from build123d import *

# Parameters (mm, degrees)
SKETCH1_W           = 250
SKETCH1_H           = 100
SKETCH2_R           = 225
BOSS_EXTRUDE1_DEPTH = 30
SKETCH3_R           = 125
BOSS_EXTRUDE2_DEPTH = 80
BOSS_EXTRUDE3_DEPTH = 10
CIRPATTERN1_COUNT   = 4


with BuildPart() as part:
    # Sketch1 → Revolve1 (revolve)
    with BuildSketch(Plane.XY, mode=Mode.PRIVATE) as revolve1_sk:
        with Locations((125, 50)):
            Rectangle(SKETCH1_W, SKETCH1_H)
    revolve(revolve1_sk.sketch.rotate(Axis((0, 0, 0), (0, 1, 0)), 90), axis=Axis((0, 0, 0), (0, 1, 0)))

    # Sketch2 → Boss-Extrude1 (add)
    with BuildSketch(Plane(origin=(0, 100, 0), x_dir=(1, 0, 0), z_dir=(0, 1, 0))):
        with Locations(Location((0, 0, 0), (0, 0, 270))):
            Circle(SKETCH2_R)
    extrude(amount=BOSS_EXTRUDE1_DEPTH)

    # Sketch3 → Boss-Extrude2 (add)
    with BuildSketch(Plane(origin=(0, 130, 0), x_dir=(1, 0, 0), z_dir=(0, 1, 0))):
        with Locations(Location((0, 0, 0), (0, 0, 270))):
            Circle(SKETCH3_R)
    extrude(amount=BOSS_EXTRUDE2_DEPTH)

    # Sketch4 → Revolve2 (revolve)
    with BuildSketch(Plane.XY):
        with BuildLine():
            Line((0, 210), (0, 275.518788168))
            ThreePointArc((0, 275.518788168), (70.565061473, 258.146319153), (125, 210))
            Line((125, 210), (0, 210))
        make_face()
    revolve(axis=Axis((0, 210, 0), (0, 1, 0)))

    # Sketch5 → Boss-Extrude3 (add, symmetric)
    with BuildSketch(Plane.XY):
        Polygon((-194.003425054, 130), (-182.358299763, 130), (-182.358299763, 145.262915146), (-182.358299763, 630), (-197.365341888, 630), (-218.16183032, 483.058469024), (-218.16183032, 211.101864805), (-194.003425054, 197.687306821), align=None)
    boss_extrude3 = extrude(amount=BOSS_EXTRUDE3_DEPTH, both=True)

    # CirPattern1: Boss-Extrude3 ×4 about axis
    cirpattern1_axis = Axis((0, 0, 0), (0, 1, 0))
    for i in range(1, CIRPATTERN1_COUNT):
        add(boss_extrude3.rotate(cirpattern1_axis, i * 360 / CIRPATTERN1_COUNT))


solid = part.part
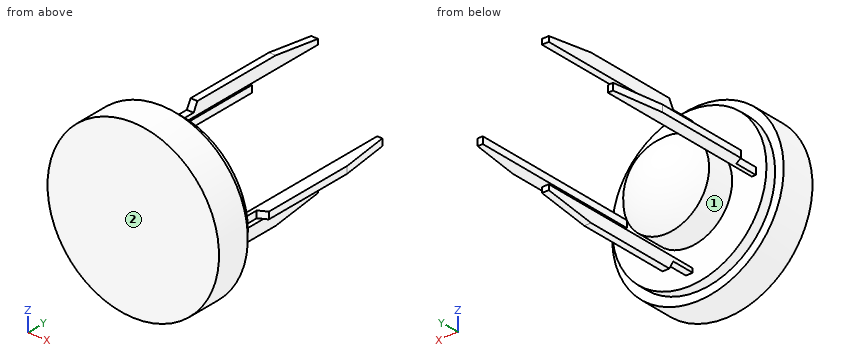
Verification items for the finished model (mm, model axes). Face numbers are marked on the shaded views. A direction names the side the tool comes from. Coordinates: 2 decimals unless noted, no trailing zeros. Write each loop counter-clockwise with the first axis right and the second up, starting at its lowest first coordinate (ties: lowest second). Pieces come first, ordered by that corner, then holes. Notation, with made-up numbers: M -19.75,44.25 L 32.25,44.25 A23 cw 32.25,53.25 Z; hole C 66,-20 d7. An arc over 180 degrees is marked long. Use CSV: the item, a comma, the result in double quotes.
Q1. Section check C-C, the plane z = 0. Enter the section's corners in (x, y).
Computed values:
outline,"M -250,0 L 250,0 L 250,100 L 225,100 L 225,130 L 194,130 L 194,197.69 L 218.16,211.1 L 218.16,483.06 L 197.37,630 L 182.36,630 L 182.36,130 L 125,130 L 125,210 A152 ccw -125,210 L -125,130 L -182.36,130 L -182.36,630 L -197.37,630 L -218.16,483.06 L -218.16,211.1 L -194,197.69 L -194,130 L -225,130 L -225,100 L -250,100 Z"
Q2. Thickness scan on line 1 along Z through (x, y) = (-5.5, 144.5); line 2 along Y through (x, z) = (220, -118); line 3 along Y through (x, z) = (28, 197.5). Record the ranges inside material, lowest first. Write a range as [from, to].
Computed values:
line 1,"[-194, -182.36], [-124.88, 124.88], [182.36, 194]"
line 2,"[0, 100]"
line 3,"[0, 130]"
Q3. Go/stop test with flat-tipped pins: P1, Ø22, axis at x = 0.5, y = 162.5, coming from the -Z side; P2, Ø10, axis at y = 347, z = -3, coming from the +X side; P3, Ø18, axis at y = 460, z = 207, coming from the -X side. Record where each tip stops, or that it passes through.
Computed values:
P1,"z = -194"
P2,"x = 218.16"
P3,"x = -10"
Q4. Set-up check for the marked faces 1 and 2: record each of +Z, -Z, +X, -X, +Y, -Y from which the full face is reachable in a straight line by a thin tool's end or side.
Computed values:
face 1,"+Y"
face 2,"+Z, -Z, +X, -X, -Y"
Q5. Section check B-B, the plane x = 0. Enter the section's corners in (y, z), and give its area (3 significant figures).
Computed values:
outline,"M 0,-250 L 100,-250 L 100,-225 L 130,-225 L 130,-194 L 197.69,-194 L 211.1,-218.16 L 483.06,-218.16 L 630,-197.37 L 630,-182.36 L 130,-182.36 L 130,-125 L 210,-125 A152 ccw 210,125 L 130,125 L 130,182.36 L 630,182.36 L 630,197.37 L 483.06,218.16 L 211.1,218.16 L 197.69,194 L 130,194 L 130,225 L 100,225 L 100,250 L 0,250 Z"
area,"124,000 mm²"
Q6. Section check D-D, the plane y = 496.5. Enter the section's corners in (x, z).
Computed values:
outline,"M -216.26,-10 L -182.36,-10 L -182.36,10 L -216.26,10 Z; M -10,-216.26 L 10,-216.26 L 10,-182.36 L -10,-182.36 Z; M -10,182.36 L 10,182.36 L 10,216.26 L -10,216.26 Z; M 182.36,-10 L 216.26,-10 L 216.26,10 L 182.36,10 Z"
Q7. Section check A-A, the plane y = 322. Enter the section's corners in (x, z), and give its area (3 significant figures).
Computed values:
outline,"M -218.16,-10 L -182.36,-10 L -182.36,10 L -218.16,10 Z; M -10,-218.16 L 10,-218.16 L 10,-182.36 L -10,-182.36 Z; M -10,182.36 L 10,182.36 L 10,218.16 L -10,218.16 Z; M 182.36,-10 L 218.16,-10 L 218.16,10 L 182.36,10 Z"
area,"2,860 mm²"
